The listing builds one solid part. Answer for the finished solid, in the listing's coordinates (mm). Face numbers are marked on the shaded views. Give positions to 0.01 mm unless a question says otherwise; leave off trailing zeros. Write each loop counter-clockwise with the first axis right and the second up, starting at its lowest first coordinate (ties: lowest second). Pieces come first, ordered by that corner, then holes. Notation, with made-up numbers: (82, 68) - (101, 68) arc R25 cw to (101, 83) - close; hole circle Ø4 at (-4.75, -8). An arc over 180 degrees is marked (long way). Return JSON: item names as keys, results as strings.
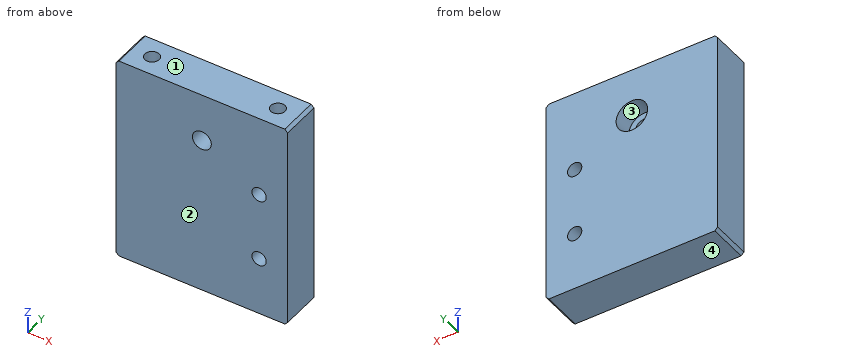
from build123d import *

# Parameters (mm, degrees)
SKETCH1_W                                            = 60
SKETCH1_H                                            = 73
BOSS_EXTRUDE1_DEPTH                                  = 7
M6_TAPPED_HOLE1_D                                    = 5
M6_TAPPED_HOLE1_DEPTH                                = 15
M6_TAPPED_HOLE1_TIP                                  = 1.502151548
M6_TAPPED_HOLE2_D                                    = 5
CHAMFER1_SIZE                                        = 1
HOLE_SIZE_PER_SOCKET_HEAD_CAP_SCREW_TYPE_D           = 6.6
HOLE_SIZE_PER_SOCKET_HEAD_CAP_SCREW_TYPE_CBORE_D     = 11
HOLE_SIZE_PER_SOCKET_HEAD_CAP_SCREW_TYPE_CBORE_DEPTH = 6.8


with BuildPart() as part:
    # Sketch1 → Boss-Extrude1 (new, symmetric)
    with BuildSketch(Plane(origin=(0, 0, 0), x_dir=(1, 0, 0), z_dir=(0, 1, 0))):
        Rectangle(SKETCH1_W, SKETCH1_H)
    extrude(amount=BOSS_EXTRUDE1_DEPTH, both=True)

    # M6 Tapped Hole1
    with Locations(Plane.XY.offset(36.5)):
        with Locations((22, 0), (-22, 0)):
            Hole(M6_TAPPED_HOLE1_D / 2, depth=M6_TAPPED_HOLE1_DEPTH)
            with Locations((0, 0, -(M6_TAPPED_HOLE1_DEPTH + M6_TAPPED_HOLE1_TIP / 2))):  # 118° drill point
                Cone(0, M6_TAPPED_HOLE1_D / 2, M6_TAPPED_HOLE1_TIP, mode=Mode.SUBTRACT)

    # M6 Tapped Hole2 (through all)
    with Locations(Plane(origin=(0, 7, 0), x_dir=(1, 0, 0), z_dir=(0, 1, 0))):
        with Locations((20, -8), (20, 16)):
            Hole(M6_TAPPED_HOLE2_D / 2)

    # Chamfer1
    chamfer1_edges = [part.edges().sort_by_distance(p)[0] for p in [
        (30, 0, 36.5),
        (-30, 0, 36.5),
        (-30, 0, -36.5),
        (30, 0, -36.5),
    ]]
    chamfer(chamfer1_edges, length=CHAMFER1_SIZE)

    # Hole Size per Socket Head Cap Screw Type1 (through all)
    with Locations(Plane(origin=(0, 7, 0), x_dir=(1, 0, 0), z_dir=(0, 1, 0))):
        with Locations((0, -19.5)):
            CounterBoreHole(HOLE_SIZE_PER_SOCKET_HEAD_CAP_SCREW_TYPE_D / 2, HOLE_SIZE_PER_SOCKET_HEAD_CAP_SCREW_TYPE_CBORE_D / 2, HOLE_SIZE_PER_SOCKET_HEAD_CAP_SCREW_TYPE_CBORE_DEPTH)


solid = part.part
Item 1: A cutting plane is placed at B-B on y = -3.75. Determine the outline of the cut face in (x, z).
Answer below:
{"outline": "(-30, -35.5) - (-29, -36.5) - (29, -36.5) - (30, -35.5) - (30, 35.5) - (29, 36.5) - (-29, 36.5) - (-30, 35.5) - close; hole circle Ø6.6 at (0, 19.5); hole circle Ø5 at (20, -16); hole circle Ø5 at (20, 8)"}
Item 2: A cutting plane is placed at C-C on x = 0. Determine the outline of the cut face in (y, z), then the cut area to 3 significant figures.
Answer below:
{"outline": "(-7, -36.5) - (7, -36.5) - (7, 14) - (0.2, 14) - (0.2, 16.2) - (-7, 16.2) - close; (-7, 22.8) - (0.2, 22.8) - (0.2, 25) - (7, 25) - (7, 36.5) - (-7, 36.5) - close", "area": "900 mm²"}
Item 3: Consider L1, parallel to X at y = 0, z = 25; L2, parallel to Z at x = 20, y = 2.75; L3, parallel to Y at x = 22, z = 33. Determine where each line is inside the solid, lowest interval first.
Answer below:
{"L1": "x = -30 to -24.5, -19.5 to 19.5, 24.5 to 30", "L2": "z = -36.5 to -18.5, -13.5 to 5.5, 10.5 to 36.5", "L3": "y = -7 to -2.5, 2.5 to 7"}
Item 4: A cutting plane is placed at D-D on z = 18. Determine the outline of the cut face in (x, y).
Answer below:
{"outline": "(-30, -7) - (-2.94, -7) - (-2.94, 0.2) - (-5.29, 0.2) - (-5.29, 7) - (-30, 7) - close; (2.94, -7) - (30, -7) - (30, 7) - (5.29, 7) - (5.29, 0.2) - (2.94, 0.2) - close"}
Item 5: The mould has two halves that part along Z. Classify the marked faces 1, 2, 3 and 4: +Z half, -Z half, draft (parallel to the pull), parting line (faces both ways), or undercut.
Answer below:
{"face 1": "+Z half", "face 2": "draft", "face 3": "undercut", "face 4": "-Z half"}
Item 6: A cutting plane is placed at A-A on z = -16. Determine the outline of the cut face in (x, y), then the cut area to 3 significant figures.
Answer below:
{"outline": "(-30, -7) - (17.5, -7) - (17.5, 7) - (-30, 7) - close; (22.5, -7) - (30, -7) - (30, 7) - (22.5, 7) - close", "area": "770 mm²"}
